```python
from build123d import *

# Parameters (mm, degrees)
SKETCH1_W           = 5
SKETCH1_H           = 15
BOSS_EXTRUDE1_DEPTH = 7
SKETCH2_W           = 20
SKETCH2_H           = 15
BOSS_EXTRUDE2_DEPTH = 2


with BuildPart() as part:
    # Sketch1 → Boss-Extrude1 (new body)
    with BuildSketch(Plane.XY):
        Rectangle(SKETCH1_W, SKETCH1_H)
    extrude(amount=BOSS_EXTRUDE1_DEPTH)

    # Sketch2 → Boss-Extrude2 (add)
    with BuildSketch(Plane.XY.offset(7)):
        with Locations((7.5, 0)):
            Rectangle(SKETCH2_W, SKETCH2_H)
    extrude(amount=BOSS_EXTRUDE2_DEPTH)


solid = part.part
```
The model under review builds one solid part; all positions refer to its coordinate system, in mm. A direction names the side the tool comes from. Coordinates: 2 decimals unless noted, no trailing zeros. Write each loop counter-clockwise with the first axis right and the second up, starting at its lowest first coordinate (ties: lowest second). Pieces come first, ordered by that corner, then holes.
1) We need section B-B on x = 15.25. State the section outline as (y, z) points.
2) To check wall thickness, follow probe 1 along X at (y, z) = (6, 1.5); probe 2 along Z at (x, y) = (10, -3). State the ranges of each line that lie inside material, in increasing order.
3) We need section C-C on z = 2.5. State the section outline as (x, y) points, then the cut area to 3 significant figures.
4) Machinability: for faces 1 (the face through (2.5, 0, 3)), 2 (the face through (-2.5, 0, 4)), which of the approach directions +Z, -Z, +X, -X, +Y, -Y give a long, thin tool a straight path to every point of the face, cutting with its end or side? Answer none if there is none.
5) We need section A-A on y = 2.25. State the section outline as (x, z) points, then the cut area to 3 significant figures.
6) Clearance check with flat-ended pins moving along their axes: pin 1 Ø4.5 at (x, y) = (10.5, -0.5) entering from -Z; pin 2 Ø1 at (x, z) = (8, 5) entering from +Y; pin 3 Ø1 at (y, z) = (-1.5, 6) entering from +X. State where each tip first meets the part, or that it passes through.
Answer list:
1. outline: (-7.5, 7) - (7.5, 7) - (7.5, 9) - (-7.5, 9) - close
2. probe 1: x = -2.5 to 2.5
2. probe 2: z = 7 to 9
3. outline: (-2.5, -7.5) - (2.5, -7.5) - (2.5, 7.5) - (-2.5, 7.5) - close
3. area: 75.0 mm2
4. face 1: -Z, +X, +Y, -Y
4. face 2: +Z, -Z, -X, +Y, -Y
5. outline: (-2.5, 0) - (2.5, 0) - (2.5, 7) - (17.5, 7) - (17.5, 9) - (-2.5, 9) - close
5. area: 75.0 mm2
6. pin 1: stops at z = 7
6. pin 2: passes through
6. pin 3: stops at x = 2.5
